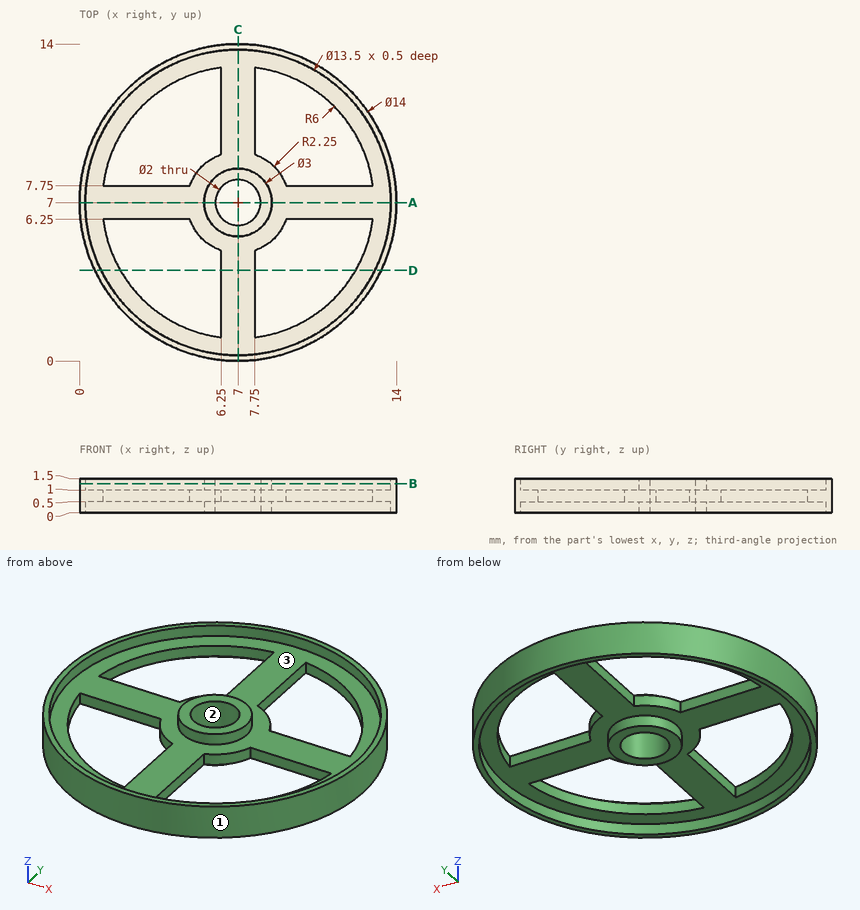
Drawing for the job (mm, zero at the part's lowest x, y, z). Round coordinates to 2 decimals unless told otherwise and drop trailing zeros. Loops run counter-clockwise (first coordinate to the right, second up) from the corner with the lowest first, then second, coordinate; pieces in that order, holes last. Notation, with made-up numbers: M 68.25,-10.75 L 74.25,-10.75 A3 ccw 74.25,-6.75 Z; hole C 45.25,22.5 d10. An arc over 180 degrees is marked long. Use a Markdown table: item, result. Add a question column.
(1) Drill centre lines: line 1 (Y direction, x = 7, z = 1.3); line 2 (Y direction, x = 10.75, z = 0.9); line 3 (X direction, y = 2.5, z = 0.7). Where is each one in solid material? Low to high.
(2) Flat gauge pins, fed straight in: pin 1 (3 mm diameter, centred on x = 8, y = 11, fed in from -Z); pin 2 (0.6 mm diameter, centred on y = 10.5, z = 0.5, fed in from +X). Where does each tip first touch, or does it go through?
(3) Cut at B-B (z = 1.3). Give the cut face in (x, y).
(4) Cut at A-A (y = 7). Give the cut face in (x, z).
(5) Cut at D-D (y = 4). Give the cut face in (x, z), and give its area (3 significant figures).
(6) Pull direction X, two halves, no side cores. Call the marked faces 1, 2 and 3: +X half, -X half, draft (parallel to the pull), parting line (faces both ways), or undercut.
Geometry says:
| question | item | result |
|---|---|---|
| 1 | line 1 | y = 0 to 0.25, 5.5 to 6, 8 to 8.5, 13.75 to 14 |
| 1 | line 2 | y = 1.09 to 2.32, 6.25 to 7.75, 11.68 to 12.91 |
| 1 | line 3 | x = 1.64 to 3.03, 6.25 to 7.75, 10.97 to 12.36 |
| 2 | pin 1 | stops at z = 0.5 |
| 2 | pin 2 | stops at x = 13.23 |
| 3 | outline | C 7,7 d14; C 7,7 d3; hole C 7,7 d13.5; hole C 7,7 d2 |
| 4 | outline | M 0,0 L 0.25,0 L 0.25,0.5 L 5.5,0.5 L 5.5,0 L 6,0 L 6,1.5 L 5.5,1.5 L 5.5,1 L 0.25,1 L 0.25,1.5 L 0,1.5 Z; M 8,0 L 8.5,0 L 8.5,0.5 L 13.75,0.5 L 13.75,0 L 14,0 L 14,1.5 L 13.75,1.5 L 13.75,1 L 8.5,1 L 8.5,1.5 L 8,1.5 Z |
| 5 | outline | M 0.68,0 L 0.95,0 L 0.95,0.5 L 1.8,0.5 L 1.8,1 L 0.95,1 L 0.95,1.5 L 0.68,1.5 Z; M 6.25,0.5 L 7.75,0.5 L 7.75,1 L 6.25,1 Z; M 12.2,0.5 L 13.05,0.5 L 13.05,0 L 13.32,0 L 13.32,1.5 L 13.05,1.5 L 13.05,1 L 12.2,1 Z |
| 5 | area | 2.43 mm² |
| 6 | face 1 | parting line |
| 6 | face 2 | undercut |
| 6 | face 3 | undercut |
